The listing builds one solid part. Answer for the finished solid, in the listing's coordinates (mm). Face numbers are marked on the shaded views. A direction names the side the tool comes from. Round coordinates to 2 decimals unless told otherwise and drop trailing zeros. Order: outer loops, then holes, each group sorted by start corner. A loop starts at its lowest first (then second) coordinate and runs counter-clockwise, first axis right, second up. Notation, with made-up numbers: (87.25, -14.5) - (123.25, -14.5) arc R28 cw to (123.25, 14.5) - close; hole circle Ø9 at (-18, 88.5). An arc over 180 degrees is marked (long way). One line per item, written item: value. Start each with the question number.
1. Section C-C, the plane y = 25.5 is taken. Give the vertices of the cut face in (x, z).
2. Section A-A, the plane x = 0 is taken. Give the vertices of the cut face in (y, z).
3. Section D-D, the plane z = 60 is taken. Give the vertices of the cut face in (x, y).
4. A tool of negligible diameter and unlimited length cuts with its end or side. For the marked faces 5, 6 and 7, from which of +Z, -Z, +X, -X, +Y, -Y can it reach the whole face along a straight path? Write none if from no direction.
5. Flat-ended cylindrical pins translate along their axes: P1, Ø24, axis at x = 80, z = 0, coming from the +Y side; P2, Ø4.5, axis at x = 89, y = 24, coming from the +Z side; P3, Ø9, axis at x = 53, y = 9, coming from the -Z side; P4, Ø1.5, axis at x = -35.5, z = 67, coming from the -Y side. Find the tip coordinate at first contact, or state that the pin passes through.
6. Straight lines are drawn through the part: line 1 (X direction, y = 5.5, z = 0); line 2 (X direction, y = 37, z = 0); line 3 (Z direction, x = 57, y = 22). For each, find the intervals that lie inside material, in ascending order.
7. Section B-B, the plane z = 0 is taken. Give the vertices of the cut face in (x, y).
8. For a pull along Z with two mould halves and no side action, classify the marked faces 1, 2, 3 and 4 as released by +Z, released by -Z, zero draft, split by the parting line, or undercut.
from build123d import *

# Parameters (mm, degrees)
HUB_PROFILE_SKETCH_R       = 40
HUB_CYLINDER_80_DEPTH      = 80
SIDE_TAB_DEPTH             = 55
ANGLED_ARM_45DEG_DEPTH     = 30
ARM_SLOT_POCKET_DEPTH      = 25
TAB_START                  = -25
TAB_SLOT_COUNTERBORE_DEPTH = 15
TAB_THROUGH_HOLE_REACH     = 142.28
HUB_START                  = 16
SKETCH1_3_R                = 30
HUB_BORE_60_DEPTH          = 64
HUB_WALL_NOTCH_REACH       = 153.834
HUB_NOTCH_SKETCH_R         = 10
HUB_NOTCH_SKETCH_R_2       = 7.5
HUB_NOTCH_SKETCH_R_3       = 20


with BuildPart() as part:
    # Hub Profile Sketch → Hub Cylinder _80 (new body)
    with BuildSketch(Plane(origin=(0, 0, 0), x_dir=(1, 0, 0), z_dir=(0, 1, 0))):
        with Locations(Location((0, 0, 0), (0, 0, 270))):
            Circle(HUB_PROFILE_SKETCH_R)
    extrude(amount=HUB_CYLINDER_80_DEPTH)

    # Arm and Tab Sketch → Side Tab (add)
    with BuildSketch(Plane(origin=(0, 0, 0), x_dir=(1, 0, 0), z_dir=(0, 1, 0))):
        with BuildLine():
            ThreePointArc((-39.757071695, -4.401732636), (-28.284271247, -28.284271247), (-4.401732636, -39.757071695))
            Line((-4.401732636, -39.757071695), (-38.890872965, -74.246212025))
            ThreePointArc((-38.890872965, -74.246212025), (-74.246212025, -74.246212025), (-74.246212025, -38.890872965))
            Line((-74.246212025, -38.890872965), (-39.757071695, -4.401732636))
        make_face()
    extrude(amount=SIDE_TAB_DEPTH)

    # Sketch3_3 → Angled Arm 45deg (add)
    with BuildSketch(Plane(origin=(0, 0, 0), x_dir=(1, 0, 0), z_dir=(0, 1, 0))):
        with BuildLine():
            ThreePointArc((23.318447633, -32.5), (40, 0), (23.318447633, 32.5))
            Line((23.318447633, 32.5), (100, 32.5))
            Line((100, 32.5), (100, -32.5))
            Line((100, -32.5), (23.318447633, -32.5))
        make_face()
    extrude(amount=ANGLED_ARM_45DEG_DEPTH)

    # Slot and Hole Sketch → Arm Slot Pocket (cut)
    with BuildSketch(Plane(origin=(0, 55, 0), x_dir=(1, 0, 0), z_dir=(0, 1, 0))):
        with BuildLine():
            Line((-44.333445626, -23.12024219), (-67.175144213, -45.961940777))
            ThreePointArc((-67.175144213, -45.961940777), (-67.175144213, -67.175144213), (-45.961940777, -67.175144213))
            Line((-45.961940777, -67.175144213), (-23.12024219, -44.333445626))
            ThreePointArc((-23.12024219, -44.333445626), (-35.355339059, -35.355339059), (-44.333445626, -23.12024219))
        make_face()
    extrude(amount=-ARM_SLOT_POCKET_DEPTH, mode=Mode.SUBTRACT)

    # Sketch4_3 → Tab Slot Counterbore (cut)
    with BuildSketch(Plane(origin=(0, 55, 0), x_dir=(1, 0, 0), z_dir=(0, 1, 0)).offset(TAB_START)):
        with BuildLine():
            Line((100, 16), (100, -16))
            Line((100, -16), (80, -16))
            ThreePointArc((80, -16), (64, 0), (80, 16))
            Line((80, 16), (100, 16))
        make_face()
    extrude(amount=-TAB_SLOT_COUNTERBORE_DEPTH, mode=Mode.SUBTRACT)

    # Sketch4_4 → Tab Through Hole (cut, up to next)
    with BuildSketch(Plane(origin=(0, 55, 0), x_dir=(1, 0, 0), z_dir=(0, 1, 0)), mode=Mode.PRIVATE) as tab_through_hole_sk1:
        with BuildLine():
            Line((16.583123952, 25), (31.224989992, 25))
            ThreePointArc((31.224989992, 25), (40, 0), (31.224989992, -25))
            Line((31.224989992, -25), (16.583123952, -25))
            ThreePointArc((16.583123952, -25), (30, 0), (16.583123952, 25))
        make_face()
    tab_through_hole_tool1 = extrude(tab_through_hole_sk1.sketch, amount=TAB_THROUGH_HOLE_REACH, mode=Mode.PRIVATE) & part.part
    add(tab_through_hole_tool1.solids().sort_by_distance((31.26913, 55, 0))[0], mode=Mode.SUBTRACT)

    # Sketch1_3 → Hub Bore _60 (cut)
    with BuildSketch(Plane(origin=(0, 0, 0), x_dir=(1, 0, 0), z_dir=(0, 1, 0)).offset(HUB_START)):
        with Locations(Location((0, 0, 0), (0, 0, 270))):
            Circle(SKETCH1_3_R)
    extrude(amount=HUB_BORE_60_DEPTH, mode=Mode.SUBTRACT)

    # Hub Notch Sketch → Hub Wall Notch (cut, up to next)
    with BuildSketch(Plane.XZ, mode=Mode.PRIVATE) as hub_wall_notch_sk1:
        with Locations(Location((-56.568542495, 56.568542495, 0), (0, 0, 270))):
            Circle(HUB_NOTCH_SKETCH_R)
    hub_wall_notch_tool1 = extrude(hub_wall_notch_sk1.sketch, amount=-HUB_WALL_NOTCH_REACH, mode=Mode.PRIVATE) & part.part
    # Hub Notch Sketch → Hub Wall Notch (cut, up to next)
    with BuildSketch(Plane.XZ, mode=Mode.PRIVATE) as hub_wall_notch_sk2:
        with Locations(Location((80, 0, 0), (0, 0, 270))):
            Circle(HUB_NOTCH_SKETCH_R_2)
    hub_wall_notch_tool2 = extrude(hub_wall_notch_sk2.sketch, amount=-HUB_WALL_NOTCH_REACH, mode=Mode.PRIVATE) & part.part
    # Hub Notch Sketch → Hub Wall Notch (cut, up to next)
    with BuildSketch(Plane.XZ, mode=Mode.PRIVATE) as hub_wall_notch_sk3:
        with Locations(Location((0, 0, 0), (0, 0, 270))):
            Circle(HUB_NOTCH_SKETCH_R_3)
    hub_wall_notch_tool3 = extrude(hub_wall_notch_sk3.sketch, amount=-HUB_WALL_NOTCH_REACH, mode=Mode.PRIVATE) & part.part
    add(hub_wall_notch_tool1.solids().sort_by_distance((-56.568542, 0, 56.568542))[0], mode=Mode.SUBTRACT)
    add(hub_wall_notch_tool2.solids().sort_by_distance((80, 0, 0))[0], mode=Mode.SUBTRACT)
    add(hub_wall_notch_tool3.solids().sort_by_distance((0, 0, 0))[0], mode=Mode.SUBTRACT)


solid = part.part
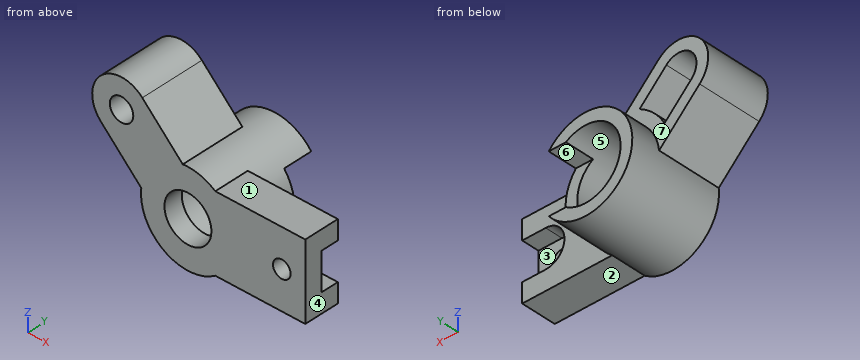
Answer list:
1. outline: (-74.25, 38.89) - (-39.76, 4.4) arc R40 ccw to (23.32, -32.5) - (100, -32.5) - (100, -16) - (80, -16) arc R16 cw to (80, 16) - (100, 16) - (100, 32.5) - (23.32, 32.5) arc R40 ccw to (-4.4, 39.76) - (-38.89, 74.25) arc R25 ccw to start; hole circle Ø20 at (-56.57, 56.57); hole circle Ø60 at (0, 0)
2. outline: (0, -40) - (80, -40) - (80, -30) - (16, -30) - (16, -20) - (0, -20) - close; (0, 20) - (16, 20) - (16, 30) - (80, 30) - (80, 40) - (0, 40) - close
3. outline: (-81.33, 0) - (-65.96, 0) - (-65.96, 30) - (-71.17, 30) - (-71.17, 55) - (-81.33, 55) - close; (-47.18, 0) - (-24.64, 0) - (-24.64, 55) - (-38.79, 55) - (-38.79, 30) - (-47.18, 30) - close
4. face 5: +Y
4. face 6: +X, +Y
4. face 7: +Z, -X, +Y
5. P1: stops at y = 15
5. P2: stops at z = 32.5
5. P3: stops at z = -32.5
5. P4: stops at y = 0
6. line 1: x = -40 to -20, 20 to 72.5, 87.5 to 100
6. line 2: x = -40 to -30, 30 to 40
6. line 3: z = -32.5 to 32.5
7. outline: (-40, 0) - (-20, 0) - (-20, 16) - (-30, 16) - (-30, 80) - (-40, 80) - close; (20, 0) - (72.5, 0) - (72.5, 15) - (64, 15) - (64, 30) - (40, 30) - (40, 55) - (30, 55) - (30, 16) - (20, 16) - close; (87.5, 0) - (100, 0) - (100, 15) - (87.5, 15) - close
8. face 1: released by +Z
8. face 2: released by -Z
8. face 3: undercut
8. face 4: zero draft
